```python
from build123d import *

# Parameters (mm, degrees)
BOSS_EXTRUDE1_DEPTH   = 750
CUT_EXTRUDE1_DEPTH    = 730
SKETCH3_W             = 246.792493201
SKETCH3_H             = 411.477698095
CUT_EXTRUDE2_DEPTH    = 1
SKETCH4_R             = 5.5
CUT_EXTRUDE3_DEPTH    = 10
M6_TAPPED_HOLE1_D     = 5
M6_TAPPED_HOLE1_DEPTH = 15
M6_TAPPED_HOLE1_TIP   = 1.502151548
M6_TAPPED_HOLE2_D     = 5
M6_TAPPED_HOLE2_DEPTH = 15
M6_TAPPED_HOLE2_TIP   = 1.502151548


with BuildPart() as part:
    # Sketch1 → Boss-Extrude1 (new body)
    with BuildSketch(Plane.XY):
        with BuildLine():
            Line((0, 0), (0, -100))
            Line((0, -100), (50, -100))
            Line((50, -100), (50, -98.925311188))
            ThreePointArc((50, -98.925311188), (48.896193111, -95.973045557), (46.126278954, -94.469104878))
            Line((46.126278954, -94.469104878), (13.317028642, -89.858065454))
            ThreePointArc((13.317028642, -89.858065454), (8.084968568, -87.017288616), (6, -81.440786869))
            Line((6, -81.440786869), (6, -18.559213131))
            ThreePointArc((6, -18.559213131), (8.084968568, -12.982711384), (13.317028642, -10.141934546))
            Line((13.317028642, -10.141934546), (46.126278954, -5.530895122))
            ThreePointArc((46.126278954, -5.530895122), (48.896193111, -4.026954443), (50, -1.074688812))
            Line((50, -1.074688812), (50, 0))
            Line((50, 0), (0, 0))
        make_face()
    extrude(amount=BOSS_EXTRUDE1_DEPTH)

    # Sketch2 → Cut-Extrude1 (cut)
    with BuildSketch(Plane(origin=(0, 0, 0), x_dir=(1, 0, 0), z_dir=(0, 1, 0))):
        Polygon((258.992644717, -472.007355283), (0, -731), (-59.777153602, -772.262203455), (30.841373369, -818.159898935), (45.044802943, -785.872759949), (459.456990019, -587.675626999), align=None)
        Polygon((25, 0), (50, -25), (50, 48.41721094), align=None)
    extrude(amount=-CUT_EXTRUDE1_DEPTH, mode=Mode.SUBTRACT)

    # Sketch3 → Cut-Extrude2 (cut)
    with BuildSketch(Plane.ZY):
        Polygon((130, 38.70177923), (130, -162.725177772), (-125.633599865, -119.606257313), (-100.418312462, 29.884375145), align=None)
        with Locations((724.396246601, 67.037069817)):
            Rectangle(SKETCH3_W, SKETCH3_H)
    extrude(amount=-CUT_EXTRUDE2_DEPTH, mode=Mode.SUBTRACT)

    # Sketch4 → Cut-Extrude3 (cut)
    with BuildSketch(Plane.ZY.offset(-1)):
        with Locations(Location((25, -30, 0), (0, 0, 270))):
            Circle(SKETCH4_R)
        with Locations(Location((105, -30, 0), (0, 0, 270))):
            Circle(SKETCH4_R)
        with Locations(Location((25, -70, 0), (0, 0, 270))):
            Circle(SKETCH4_R)
        with Locations(Location((105, -70, 0), (0, 0, 270))):
            Circle(SKETCH4_R)
        with Locations(Location((626, -30, 0), (0, 0, 270))):
            Circle(SKETCH4_R)
        with Locations(Location((706, -70, 0), (0, 0, 270))):
            Circle(SKETCH4_R)
        with Locations(Location((626, -70, 0), (0, 0, 270))):
            Circle(SKETCH4_R)
        with Locations(Location((706, -30, 0), (0, 0, 270))):
            Circle(SKETCH4_R)
    extrude(amount=-CUT_EXTRUDE3_DEPTH, mode=Mode.SUBTRACT)

    # M6 Tapped Hole1
    with Locations(Plane(origin=(0, -100, 0), x_dir=(-1, 0, 0), z_dir=(0, -1, 0))):
        with Locations((-21.5, -12.5)):
            Hole(M6_TAPPED_HOLE1_D / 2, depth=M6_TAPPED_HOLE1_DEPTH)
            with Locations((0, 0, -(M6_TAPPED_HOLE1_DEPTH + M6_TAPPED_HOLE1_TIP / 2))):  # 118° drill point
                Cone(0, M6_TAPPED_HOLE1_D / 2, M6_TAPPED_HOLE1_TIP, mode=Mode.SUBTRACT)

    # M6 Tapped Hole2
    with Locations(Plane(origin=(0, -100, 0), x_dir=(-1, 0, 0), z_dir=(0, -1, 0))):
        with Locations((-21.5, -132.5)):
            Hole(M6_TAPPED_HOLE2_D / 2, depth=M6_TAPPED_HOLE2_DEPTH)
            with Locations((0, 0, -(M6_TAPPED_HOLE2_DEPTH + M6_TAPPED_HOLE2_TIP / 2))):  # 118° drill point
                Cone(0, M6_TAPPED_HOLE2_D / 2, M6_TAPPED_HOLE2_TIP, mode=Mode.SUBTRACT)


solid = part.part
```
Geometry check sheet. Reference: the model listing, model coordinates, mm. A direction names the side the tool comes from. Give positions to 0.01 mm unless a question says otherwise; leave off trailing zeros. Order: outer loops, then holes, each group sorted by start corner. A loop starts at its lowest first (then second) coordinate and runs counter-clockwise, first axis right, second up. Notation, with made-up numbers: (26, 63.25) - (43, 63.25) arc R24 ccw to (43, 77.25) - close; hole circle Ø11 at (-5.5, 13). An arc over 180 degrees is marked (long way). Write item = value, one per line. Start each with the question number.
1) Section check B-B (z = 381). Enter the section's corners in (x, y).
2) Draft check along Y on faces 4 (the flat face through (25, -100, 360)), 5 (the flat face through (6, -50, 357)), 6 (the flat face through (5, -49, 0)). Enter one of: released by +Y, released by -Y, zero draft, split by the parting line, or undercut.
3) Gauge pin test, flat ends, axial feed: pin 1 Ø17.5 at (y, z) = (-70, 706) entering from -X; pin 2 Ø10 at (y, z) = (-70, 25) entering from -X; pin 3 Ø8 at (y, z) = (-18.5, 270) entering from +X; pin 4 Ø10 at (x, y) = (5, -88) entering from +Z. Record the tip position at first contact, or that the pin passes through.
4) Access from +Z, -Z, +X, -X, +Y, -Y to the whole of each face (thin tool, end or side, straight path). Record for faces 1 (the flat face through (1, -49, 66)), 2 (the flat face through (1, -49, 665)), 3 (the flat face through (29.49, -7.87, 353.82)).
5) Scan lines: L1, parallel to Y at x = 3, z = 706; L2, parallel to Z at x = 2, y = -30; L3, parallel to Z at x = 3.75, y = -70. Record each from-to range of solid material in increasing order.
6) Section check A-A (z = 76). Enter the section's corners in (x, y).
Geometry check:
q1.outline = (0, -100) - (50, -100) - (50, -98.93) arc R4.5 ccw to (46.13, -94.47) - (13.32, -89.86) arc R8.5 cw to (6, -81.44) - (6, -18.56) arc R8.5 cw to (13.32, -10.14) - (46.13, -5.53) arc R4.5 ccw to (50, -1.07) - (50, 0) - (0, 0) - close
q2.face_4 = released by -Y
q2.face_5 = undercut
q2.face_6 = zero draft
q3.pin_1 = 1
q3.pin_2 = through
q3.pin_3 = 7.03
q3.pin_4 = 730
q4.face_1 = -Z, -X, +Y, -Y
q4.face_2 = +Z, -X, +Y, -Y
q4.face_3 = +Z, -Z, +X
q5.L1 = -100 to -75.5, -64.5 to -35.5, -24.5 to 0
q5.L2 = 0 to 19.5, 30.5 to 99.5, 110.5 to 620.5, 631.5 to 700.5, 711.5 to 729
q5.L3 = 0 to 19.5, 30.5 to 99.5, 110.5 to 620.5, 631.5 to 700.5, 711.5 to 727.25
q6.outline = (1, -100) - (50, -100) - (50, -98.93) arc R4.5 ccw to (46.13, -94.47) - (13.32, -89.86) arc R8.5 cw to (6, -81.44) - (6, -18.56) arc R8.5 cw to (13.32, -10.14) - (46.13, -5.53) arc R4.5 ccw to (50, -1.07) - (50, 0) - (1, 0) - close
